from build123d import *

# Parameters (mm, degrees)
BASE_BLOCK_DEPTH       = 32
SLOT_CUT_DEPTH         = 140
ANGLED_WING_DEPTH      = 40
WING_TRIM_CUT_SKETCH_R = 10
WING_TRIM_CUT_DEPTH    = 40


with BuildPart() as part:
    # Base Block Sketch → Base Block (new body)
    with BuildSketch(Plane.XY):
        Polygon((75, 85), (150, 0), (0, 0), (0, 85), align=None)
    extrude(amount=-BASE_BLOCK_DEPTH)

    # Slot Cut Sketch → Slot Cut (cut)
    with BuildSketch(Plane(origin=(84.338521401, 74.416342412, 0), x_dir=(0, 0, -1), z_dir=(0.7498378553650925, 0.6616216370868463, 0))):
        Polygon((24, -22.564325319), (32, -22.564325319), (32, -62.564325319), (24, -62.564325319), (24, -72.564325319), (8, -72.564325319), (8, -12.564325319), (24, -12.564325319), align=None)
    extrude(amount=-SLOT_CUT_DEPTH, mode=Mode.SUBTRACT)

    # Angled Wing Sketch → Angled Wing (add)
    with BuildSketch(Plane.XY):
        Polygon((120.39128367, 33.556545174), (118.82693902, 23.679661768), (0, 42.5), (1.56434465, 52.376883406), align=None)
    extrude(amount=ANGLED_WING_DEPTH)

    # Wing Trim Cut Sketch → Wing Trim Cut (cut)
    with BuildSketch(Plane(origin=(8.130955781, 51.336834377, 0), x_dir=(0.9876883405951389, -0.15643446504022435, 0), z_dir=(0.15643446504022435, 0.9876883405951389, 0))):
        with Locations(Location((43.351535236, -22, 0), (0, 0, 180))):
            Circle(WING_TRIM_CUT_SKETCH_R)
        Polygon((-6.648464764, 0), (20.17251839, -46.455305531), (-6.648464764, -46.455305531), align=None)
        Polygon((113.659666997, -15), (81.480803865, -47.178863132), (138.076260789, -47.178863132), align=None)
    extrude(amount=-WING_TRIM_CUT_DEPTH, mode=Mode.SUBTRACT)


solid = part.part
Source: CAD feature listing. Evaluate the final solid. Frame: model axes, mm. A direction names the side the tool comes from. Round coordinates to 2 decimals unless told otherwise and drop trailing zeros. Loops run counter-clockwise (first coordinate to the right, second up) from the corner with the lowest first, then second, coordinate; pieces in that order, holes last. Notation, with made-up numbers: (77, 33.25) - (104, 33.25) arc R14 cw to (104, 47.25) - close; hole circle Ø5 at (44, -2). An arc over 180 degrees is marked (long way). Write item = value, one per line. Start each with the question number.
Item 1: First-contact query: pin 1 Ø4 at (x, y) = (49, 13.5) entering from +Z; pin 2 Ø6 at (x, z) = (88.5, -20.5) entering from -Y; pin 3 Ø6 at (x, z) = (94.5, 24.5) entering from -Y. Flat tips, straight axial feed; report the tip coordinate or a pass-through.
Item 2: Mould query, pull axis Z, two halves, no side actions, for faces 4 (the face through (39, 43, -32)), 5 (the face through (110.365, 13.944, -28.056)), 6 (the face through (80, 22, -8)). Classes: released by +Z, released by -Z, zero draft, split by the parting line, or undercut.
Item 3: Reachability of faces 1 (the face through (119.62, 28.69, 7.4)), 2 (the face through (60.146, 43.098, 15.276)), 3 (the face through (60, 29, -24)) from +Z, -Z, +X, -X, +Y, -Y: full face, straight path, thin tool, end or side. Return the list, or none.
Item 4: Section query B-B on y = 76.5. Output: boundary loops of the cut face in (x, z).
Item 5: Section query D-D on z = 26.5. Output: boundary loops of the cut face in (x, y).
Item 6: Section query C-C on x = 128. Output: boundary loops of the cut face in (y, z), plus the area to 3 significant figures.
Item 7: Section query A-A on z = -21.5. Output: boundary loops of the cut face in (x, y).
Item 8: Material intervals for line 1 (Z direction, x = 34, y = 8.5); line 2 (Z direction, x = 51, y = 7); line 3 (X direction, y = 5, z = -16), sorted ascending.
Results list:
q1.pin_1 = 0
q1.pin_2 = 58.69
q1.pin_3 = 27.06
q2.face_4 = released by -Z
q2.face_5 = zero draft
q2.face_6 = undercut
q3.face_1 = +Z, +X, -Y
q3.face_2 = +Z, +X, +Y
q3.face_3 = -Y
q4.outline = (0, -32) - (82.5, -32) - (82.5, 0) - (0, 0) - close
q5.outline = (15.11, 40.11) - (40.56, 36.08) - (42.13, 45.95) - (16.68, 49.98) - close; (58.2, 33.28) - (107.47, 25.48) - (109.03, 35.36) - (59.77, 43.16) - close
q6.outline = (0, -32) - (24.93, -32) - (24.93, -24) - (16.17, -24) - (16.17, -8) - (24.93, -8) - (24.93, 0) - (0, 0) - close
q6.area = 658 mm²
q7.outline = (0, 0) - (18.99, 0) - (92.65, 65) - (75, 85) - (0, 85) - close; (109.68, 0) - (150, 0) - (132.35, 20) - close
q8.line_1 = -32 to -24, -8 to 0
q8.line_2 = -8 to 0
q8.line_3 = 0 to 24.66, 115.34 to 145.59
